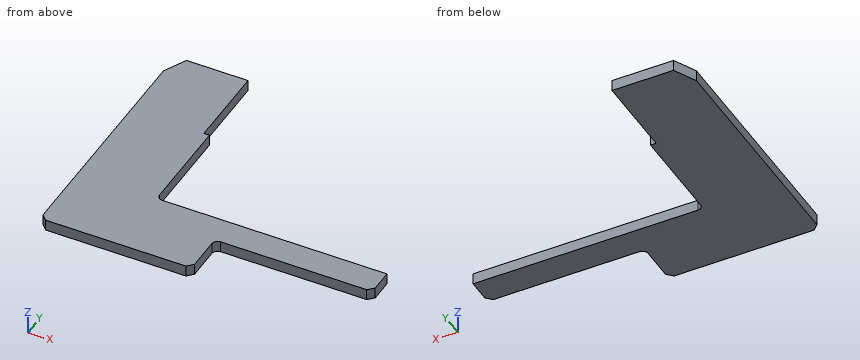
```python
from build123d import *

# Parameters (mm, degrees)
BOSS_EXTRUDE1_DEPTH = 40
CHAMFER1_SIZE       = 20
FILLET1_R           = 20


with BuildPart() as part:
    # Sketch1 → Boss-Extrude1 (new body)
    with BuildSketch(Plane.XY):
        Polygon((-572.578678855, 758.246779508), (-572.578678855, -80.753220492), (-33.578678855, -80.753220492), (-33.578678855, 78.246779508), (526.421321145, 78.246779508), (526.421321145, 178.246779508), (-293.578678855, 178.246779508), (-293.578678855, 538.246779508), (-313.578678855, 538.246779508), (-313.578678855, 838.246779508), (-532.578678855, 838.246779508), align=None)
    extrude(amount=BOSS_EXTRUDE1_DEPTH)

    # Chamfer1
    chamfer1_edges = [part.edges().sort_by_distance(p)[0] for p in [
        (-572.578678855, -80.753220492, 20),
        (526.421321145, 78.246779508, 20),
        (-33.578678855, -80.753220492, 20),
    ]]
    chamfer(chamfer1_edges, length=CHAMFER1_SIZE)

    # Fillet1
    fillet1_edges = [part.edges().sort_by_distance(p)[0] for p in [
        (-293.578678855, 178.246779508, 20),
        (-33.578678855, 78.246779508, 20),
    ]]
    fillet(fillet1_edges, radius=FILLET1_R)


solid = part.part
```
Geometry: final body of the model. Coordinates: model frame, mm. Give positions to 0.01 mm unless a question says otherwise; leave off trailing zeros. Loops run counter-clockwise (first coordinate to the right, second up) from the corner with the lowest first, then second, coordinate; pieces in that order, holes last. Notation, with made-up numbers: (13.5, 65) -> (56.5, 65) arc R23 cw to (56.5, 93) -> close; hole circle Ø3 at (78.25, -0.75). An arc over 180 degrees is marked (long way). Return JSON: item names as keys, results as strings.
Item 1: Section A-A, the plane z = 17. Output: boundary loops of the cut face in (x, y), plus the area to 3 significant figures.
Filled in:
{"outline": "(-572.58, -60.75) -> (-552.58, -80.75) -> (-53.58, -80.75) -> (-33.58, -60.75) -> (-33.58, 58.25) arc R20 cw to (-13.58, 78.25) -> (506.42, 78.25) -> (526.42, 98.25) -> (526.42, 178.25) -> (-273.58, 178.25) arc R20 cw to (-293.58, 198.25) -> (-293.58, 538.25) -> (-313.58, 538.25) -> (-313.58, 838.25) -> (-532.58, 838.25) -> (-572.58, 758.25) -> close", "area": "372,000 mm^2"}
Item 2: Line query: line 1 (Y direction, x = 338, z = 14); line 2 (X direction, y = 41.5, z = 23); line 3 (Y direction, x = -197, z = 28.5). Output: solid intervals per line, ascending.
Filled in:
{"line 1": "78.25 to 178.25", "line 2": "-572.58 to -33.58", "line 3": "-80.75 to 178.25"}
Item 3: Section C-C, the plane y = 693.5. Output: boundary loops of the cut face in (x, z).
Filled in:
{"outline": "(-572.58, 0) -> (-313.58, 0) -> (-313.58, 40) -> (-572.58, 40) -> close"}
Item 4: Pin query (flat end, axial travel): P1, Ø6, axis at x = -307.5, z = 30, coming from the +Y side; P2, Ø8, axis at x = 347, z = 20, coming from the -Y side; P3, Ø10, axis at x = 277, z = 14, coming from the +Y side. Return the tip coordinate at first contact, or that it passes through.
Filled in:
{"P1": "y = 538.25", "P2": "y = 78.25", "P3": "y = 178.25"}
Item 5: Section B-B, the plane x = 66.5. Output: boundary loops of the cut face in (y, z).
Filled in:
{"outline": "(78.25, 0) -> (178.25, 0) -> (178.25, 40) -> (78.25, 40) -> close"}
